Geometry check sheet. Reference: drawing and pictorial views, mm from the part's lowest x, y, z. Coordinates: 2 decimals unless noted, no trailing zeros. Loops run counter-clockwise (first coordinate to the right, second up) from the corner with the lowest first, then second, coordinate; pieces in that order, holes last.
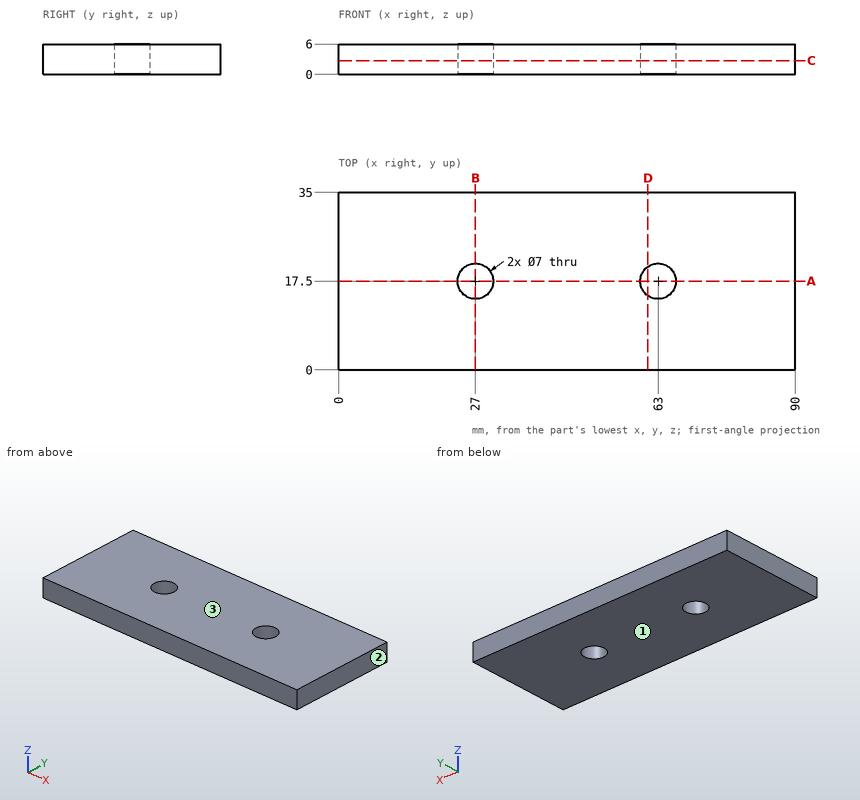
1) Section check D-D on x = 61. Record the cut outline in (y, z), and give its area (3 significant figures).
Data:
outline: (0, 0) - (14.63, 0) - (14.63, 6) - (0, 6) - close; (20.37, 0) - (35, 0) - (35, 6) - (20.37, 6) - close
area: 176 mm2
2) Section check C-C on z = 2.7. Record the cut outline in (x, y), and give its area (3 significant figures).
Data:
outline: (0, 0) - (90, 0) - (90, 35) - (0, 35) - close; hole circle Ø7 at (27, 17.5); hole circle Ø7 at (63, 17.5)
area: 3,070 mm2
3) Section check A-A on y = 17.5. Record the cut outline in (x, z), and give its area (3 significant figures).
Data:
outline: (0, 0) - (23.5, 0) - (23.5, 6) - (0, 6) - close; (30.5, 0) - (59.5, 0) - (59.5, 6) - (30.5, 6) - close; (66.5, 0) - (90, 0) - (90, 6) - (66.5, 6) - close
area: 456 mm2
4) Mould release check, pull along Z, two halves, no side actions. Record for the marked faces 1, 2 and 3: +Z half, -Z half, draft (parallel to the pull), parting line (faces both ways), or undercut.
Data:
face 1: -Z half
face 2: draft
face 3: +Z half
5) Section check B-B on x = 27. Record the cut outline in (y, z).
Data:
outline: (0, 0) - (14, 0) - (14, 6) - (0, 6) - close; (21, 0) - (35, 0) - (35, 6) - (21, 6) - close
6) Material ranges on probe 1 along Y at (x, z) = (63, 1.65); probe 2 along X at (y, z) = (17, 1.45); probe 3 along Y at (x, z) = (25.5, 1.7), recorded low to high.
Data:
probe 1: y = 0 to 14, 21 to 35
probe 2: x = 0 to 23.54, 30.46 to 59.54, 66.46 to 90
probe 3: y = 0 to 14.34, 20.66 to 35
